The model under review builds one solid part; all positions refer to its coordinate system, in mm. Face numbers are marked on the shaded views. A direction names the side the tool comes from. Give positions to 0.01 mm unless a question says otherwise; leave off trailing zeros. Loops run counter-clockwise (first coordinate to the right, second up) from the corner with the lowest first, then second, coordinate; pieces in that order, holes last. Notation, with made-up numbers: M 25.5,28 L 47.5,28 A15 cw 47.5,39 Z; hole C 27,40.25 d10. An arc over 180 degrees is marked long. Write item = value, one per line. Start each with the question number.
1. We need section A-A on z = 0. Give the boundary of the cut face in (x, y), then the cut area to 3 significant figures.
2. For pin 1 (3 mm diameter, centred on y = 3.5, z = -2.5, fed in from +X); pin 2 (1.5 mm diameter, centred on x = 1, z = 0, fed in from +Y), all flat-tipped, find the tip position at first contact; note any pin that passes through.
3. We need section D-D on y = 1.15. Give the boundary of the cut face in (x, z), then the cut area to 3 significant figures.
4. We need section B-B on x = 0. Give the boundary of the cut face in (y, z).
5. Draft analysis for pull direction Y (two halves, no side actions). For the marked faces 3, 4 and 5, state which applies: pulls with the +Y half, pulls with the -Y half, needs draft (parallel to the pull), parting line crosses it, or undercut.
6. Wall thickness on line 1 along Y through (x, z) = (2.5, 4.75); line 2 along X through (y, z) = (2.55, 0); line 3 along X through (y, z) = (1.1, -2): over which ranges is each line inside the solid? List them lowest first. Write a range as from..to.
7. We need section C-C on y = 1.9. Give the boundary of the cut face in (x, z).
8. For the marked faces 1 and 2, list the 3-axis set-ups (+Z, -Z, +X, -X, +Y, -Y) from which the entire face can be reached by the end or side of a thin tool; tool diameter is ignored.
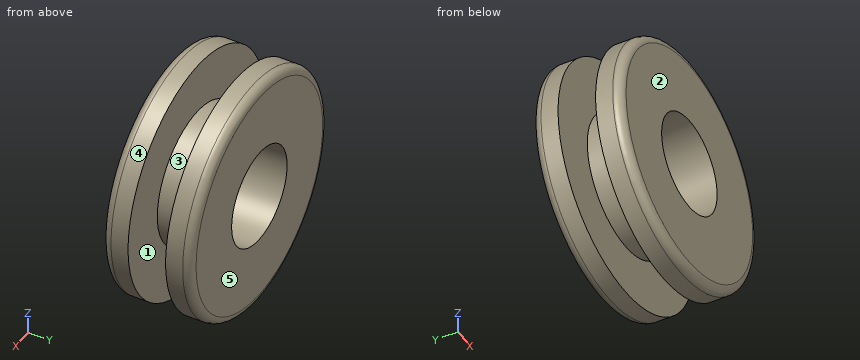
from build123d import *


with BuildPart() as part:
    # 草图1 → 旋转1 (revolve)
    with BuildSketch(Plane.XY, mode=Mode.PRIVATE) as revolve_1_sk:
        with BuildLine():
            Line((2.85, 5.2), (6.5, 5.2))
            ThreePointArc((6.5, 5.2), (6.853553391, 5.053553391), (7, 4.7))
            Line((7, 4.7), (7, 3.7))
            Line((7, 3.7), (4, 3.7))
            Line((4, 3.7), (4, 1.5))
            Line((4, 1.5), (7, 1.5))
            Line((7, 1.5), (7, 0.5))
            ThreePointArc((7, 0.5), (6.853553391, 0.146446609), (6.5, 0))
            Line((6.5, 0), (2.85, 0))
            Line((2.85, 0), (2.85, 5.2))
        make_face()
    revolve(revolve_1_sk.sketch.rotate(Axis((0, 0, 0), (0, 1, 0)), 90), axis=Axis((0, 0, 0), (0, 1, 0)))


solid = part.part
Final values:
q1.outline = M -7,0.5 A0.5 ccw -6.5,0 L -2.85,0 L -2.85,5.2 L -6.5,5.2 A0.5 ccw -7,4.7 L -7,3.7 L -4,3.7 L -4,1.5 L -7,1.5 Z; M 2.85,0 L 6.5,0 A0.5 ccw 7,0.5 L 7,1.5 L 4,1.5 L 4,3.7 L 7,3.7 L 7,4.7 A0.5 ccw 6.5,5.2 L 2.85,5.2 Z
q1.area = 29.7 mm²
q2.pin_1 = 6.93
q2.pin_2 = through
q3.outline = C 0,0 d14; hole C 0,0 d5.7
q3.area = 128 mm²
q4.outline = M 0,-6.5 A0.5 ccw 0.5,-7 L 1.5,-7 L 1.5,-4 L 3.7,-4 L 3.7,-7 L 4.7,-7 A0.5 ccw 5.2,-6.5 L 5.2,-2.85 L 0,-2.85 Z; M 0,2.85 L 5.2,2.85 L 5.2,6.5 A0.5 ccw 4.7,7 L 3.7,7 L 3.7,4 L 1.5,4 L 1.5,7 L 0.5,7 A0.5 ccw 0,6.5 Z
q5.face_3 = undercut
q5.face_4 = needs draft
q5.face_5 = pulls with the +Y half
q6.line_1 = 0..1.5, 3.7..5.2
q6.line_2 = -4..-2.85, 2.85..4
q6.line_3 = -6.71..-2.03, 2.03..6.71
q7.outline = C 0,0 d8; hole C 0,0 d5.7
q8.face_1 = none
q8.face_2 = +Z, -Z, +X, -X, -Y
